Verification items for the finished model (mm, model axes). A direction names the side the tool comes from. Give positions to 0.01 mm unless a question says otherwise; leave off trailing zeros. Order: outer loops, then holes, each group sorted by start corner. A loop starts at its lowest first (then second) coordinate and runs counter-clockwise, first axis right, second up. Notation, with made-up numbers: M 21.25,54 L 54.25,54 A19 ccw 54.25,85 Z; hole C -39.75,27 d2. An arc over 180 degrees is marked long. Answer as a JSON object with one key per item and string values.
```python
from build123d import *

# Parameters (mm, degrees)
SKETCH_1_W             = 26
SKETCH_1_H             = 80
EXTRUDE_1_DEPTH        = 10
SKETCH_2_R             = 8.1
CUT_EXTRUDE_1_DEPTH    = 44.231932642
EXTRUDE_2_DEPTH        = 10
CHAMFER_1_SIZE         = 2
CHAMFER_2_SIZE         = 2
SKETCH_9_R             = 11
CUT_EXTRUDE_2_DEPTH    = 2
HOLE_WIZARD_M4_1_D     = 3.3
HOLE_WIZARD_M4_1_DEPTH = 10.1
HOLE_WIZARD_M4_1_TIP   = 0.991420021


with BuildPart() as part:
    # 草图1 → 凸台-拉伸1 (new body)
    with BuildSketch(Plane.XY):
        Rectangle(SKETCH_1_W, SKETCH_1_H)
    extrude(amount=EXTRUDE_1_DEPTH)

    # 草图2 → 切除-拉伸1 (cut, through all)
    with BuildSketch(Plane.XY.offset(10)):
        Circle(SKETCH_2_R)
    extrude(amount=-CUT_EXTRUDE_1_DEPTH, mode=Mode.SUBTRACT)

    # 草图7 → 凸台-拉伸2 (add)
    with BuildSketch(Plane(origin=(0, 40, 0), x_dir=(1, 0, 0), z_dir=(0, 1, 0))):
        Polygon((13, -10), (13, -15), (-8, -22), (-13, -22), (-13, -10), align=None)
    extrude_2 = extrude(amount=-EXTRUDE_2_DEPTH)

    # 镜向1: 凸台-拉伸2 across plane
    add(extrude_2.mirror(Plane.ZX))

    # 倒角1
    chamfer_1_edges = [part.edges().sort_by_distance(p)[0] for p in [
        (13, -40, 7.5),
        (13, 40, 7.5),
    ]]
    chamfer(chamfer_1_edges, length=CHAMFER_1_SIZE)

    # 倒角2
    chamfer_2_edges = [part.edges().sort_by_distance(p)[0] for p in [
        (-1, -40, 0),
        (-1, 40, 0),
    ]]
    chamfer(chamfer_2_edges, length=CHAMFER_2_SIZE)

    # 草图9 → 切除-拉伸2 (cut)
    with BuildSketch(Plane(origin=(0, 0, 10), x_dir=(-1, 0, 0), z_dir=(0, 0, -1))):
        Circle(SKETCH_9_R)
    extrude(amount=CUT_EXTRUDE_2_DEPTH, mode=Mode.SUBTRACT)

    # M4 螺纹孔1
    with Locations(Plane.ZY.offset(13)):
        with Locations((17, 35), (7, 35), (7, -35), (17, -35)):
            Hole(HOLE_WIZARD_M4_1_D / 2, depth=HOLE_WIZARD_M4_1_DEPTH)
            with Locations((0, 0, -(HOLE_WIZARD_M4_1_DEPTH + HOLE_WIZARD_M4_1_TIP / 2))):  # 118° drill point
                Cone(0, HOLE_WIZARD_M4_1_D / 2, HOLE_WIZARD_M4_1_TIP, mode=Mode.SUBTRACT)


solid = part.part
```
Q1. Material ranges on L1, parallel to Z at x = -10.75, y = 35; L2, parallel to Y at x = -10.5, z = 7; L3, parallel to Y at x = -0.75, z = 11, recorded low to high.
Resolved:
{"L1": "z = 0 to 5.35, 8.65 to 15.35, 18.65 to 22", "L2": "y = -40 to -36.65, -33.35 to 33.35, 36.65 to 40", "L3": "y = -40 to -30, 30 to 40"}
Q2. Section check B-B on z = 19.5. Record the cut outline in (x, y), then the cut area to 3 significant figures.
Resolved:
{"outline": "M -13,-40 L -0.5,-40 L -0.5,-30 L -13,-30 Z; M -13,30 L -0.5,30 L -0.5,40 L -13,40 Z", "area": "250 mm²"}
Q3. Section check C-C on x = 0. Record the cut outline in (y, z).
Resolved:
{"outline": "M -40,2 L -38,0 L -8.1,0 L -8.1,8 L -11,8 L -11,10 L -30,10 L -30,19.33 L -40,19.33 Z; M 8.1,0 L 38,0 L 40,2 L 40,19.33 L 30,19.33 L 30,10 L 11,10 L 11,8 L 8.1,8 Z"}
Q4. Section check A-A on y = 0. Record the cut outline in (x, z).
Resolved:
{"outline": "M -13,0 L -8.1,0 L -8.1,8 L -11,8 L -11,10 L -13,10 Z; M 8.1,0 L 13,0 L 13,10 L 11,10 L 11,8 L 8.1,8 Z"}
Q5. Tool access check on faces 1 (the face through (2.38, -10.74, 9.01)), 2 (the face through (-3, -30, 15)), 3 (the face through (-7.879, 36.115, 8.216)). Record the directions out of +Z, -Z, +X, -X, +Y, -Y that give a thin tool (end or side, any length) a straight path to the whole face; none if there is none.
Resolved:
{"face 1": "+Z", "face 2": "+Z, +X, -X", "face 3": "-X"}
Q6. Release check for a two-part mould opening along X. For faces 4 (the face through (4.1, -7.3, 8)), 5 (the face through (-7.879, -33.885, 8.216)), 6 (the face through (-2.1, 34.7, 7.1)) record: +X half, -X half, draft (parallel to the pull), parting line (faces both ways), or undercut.
Resolved:
{"face 4": "undercut", "face 5": "draft", "face 6": "-X half"}
Q7. Section check D-D on x = -7.25. Record the cut outline in (y, z).
Resolved:
{"outline": "M -40,2 L -38,0 L -3.61,0 L -3.61,8 L -8.27,8 L -8.27,10 L -30,10 L -30,21.75 L -40,21.75 Z; M 3.61,0 L 38,0 L 40,2 L 40,21.75 L 30,21.75 L 30,10 L 8.27,10 L 8.27,8 L 3.61,8 Z; hole C -35,7 d3.3; hole C -35,17 d3.3; hole C 35,7 d3.3; hole C 35,17 d3.3"}
Q8. Gauge pin test, flat ends, axial feed: pin 1 Ø2 at (x, y) = (3, -5.5) entering from +Z; pin 2 Ø5.5 at (y, z) = (-35, 17) entering from -X; pin 3 Ø8 at (x, y) = (3.5, -5) entering from +Z; pin 4 Ø8 at (x, y) = (-4.5, 13) entering from +Z. Record the tip position at first contact, or that the pin passes through.
Resolved:
{"pin 1": "passes through", "pin 2": "stops at x = -13", "pin 3": "stops at z = 8", "pin 4": "stops at z = 10"}
